Read the model definition and answer for the solid it produces. Units are mm, in the model's axes. A direction names the side the tool comes from. Give positions to 0.01 mm unless a question says otherwise; leave off trailing zeros. Write each loop counter-clockwise with the first axis right and the second up, starting at its lowest first coordinate (ties: lowest second). Pieces come first, ordered by that corner, then holes. Notation, with made-up numbers: M -23,-9 L 7,-9 A29 cw 7,22 Z; hole C 29.5,-27.5 d7. An arc over 180 degrees is marked long. Use a Markdown table: item, result. Add a question column.
Item 1: For faces 4 (the flat face through (-28, -25, 6.4)), 5 (the flat face through (0, 1, 0)), determine the directions among +Z, -Z, +X, -X, +Y, -Y from which every point of the face is accessible in a straight line to the end or side of a thin tool.
Item 2: A cutting plane is placed at B-B on y = -21. Determine the outline of the cut face in (x, z).
Item 3: A cutting plane is placed at D-D on y = -33. Determine the outline of the cut face in (x, z), then the cut area to 3 significant figures.
Item 4: A cutting plane is placed at C-C on z = 2.5. Count the separate pieces of the cut face and the enclosed holes in it, then the cut area to 3 significant figures.
Item 5: Consider probe 1 along Y at (x, z) = (28, 8.65); probe 2 along Y at (x, z) = (-28, 3); probe 3 along X at (y, z) = (19, 3.25). Determine where each line is inside the solid, lowest interval first. Write a range as [from, to].
Item 6: Given P1, Ø4.5, axis at x = 28, y = -33, coming from the -Z side; P2, Ø3.5, axis at x = -26, y = 22.5, coming from the -Z side; P3, Ø12, axis at x = 26, y = 19.5, coming from the -Z side, each flat-ended and moving along its own axis, determine where each tip first touches the part or whether it passes through.
Item 7: The mould has two halves that part along Y. Classify faces 1 (the flat face through (0, 1, 12)), 2 (the cylindrical face through (27.67, -30.52, 6.08)), 3 (the flat face through (0, -40, 6)): pulls with the +Y half, pulls with the -Y half, needs draft (parallel to the pull), parting line crosses it, or undercut.
Item 8: A cutting plane is placed at A-A on x = 28. Determine the outline of the cut face in (y, z), then the cut area to 3 significant figures.
from build123d import *

# Parameters (mm, degrees)
SKETCH_1_W                     = 70
SKETCH_1_H                     = 80
EXTRUDE_1_DEPTH                = 12
HOLE_WIZARD_M6_1_D             = 5
HOLE_WIZARD_M6_1_2_D           = 6.6
HOLE_WIZARD_M6_1_2_CBORE_D     = 11
HOLE_WIZARD_M6_1_2_CBORE_DEPTH = 6.4


with BuildPart() as part:
    # 草图1 → 凸台-拉伸1 (new body)
    with BuildSketch(Plane.XY):
        Rectangle(SKETCH_1_W, SKETCH_1_H)
    extrude(amount=EXTRUDE_1_DEPTH)

    # Hole Wizard M6 _1 (through all)
    with Locations(Plane(origin=(0, 0, 0), x_dir=(-1, 0, 0), z_dir=(0, 0, -1))):
        with Locations((28, 33), (28, -33), (-28, -33), (-28, 33)):
            Hole(HOLE_WIZARD_M6_1_D / 2)

    # Hole Wizard M6 _1 2 (through all)
    with Locations(Plane(origin=(0, 0, 0), x_dir=(-1, 0, 0), z_dir=(0, 0, -1))):
        with Locations((-28, -21), (-28, 21), (28, -21), (28, 21)):
            CounterBoreHole(HOLE_WIZARD_M6_1_2_D / 2, HOLE_WIZARD_M6_1_2_CBORE_D / 2, HOLE_WIZARD_M6_1_2_CBORE_DEPTH)


solid = part.part
Filled in:
| question | item | result |
|---|---|---|
| 1 | face 4 | -Z |
| 1 | face 5 | -Z, +X, -X, +Y, -Y |
| 2 | outline | M -35,0 L -33.5,0 L -33.5,6.4 L -31.3,6.4 L -31.3,12 L -35,12 Z; M -24.7,6.4 L -22.5,6.4 L -22.5,0 L 22.5,0 L 22.5,6.4 L 24.7,6.4 L 24.7,12 L -24.7,12 Z; M 31.3,6.4 L 33.5,6.4 L 33.5,0 L 35,0 L 35,12 L 31.3,12 Z |
| 3 | outline | M -35,0 L -30.5,0 L -30.5,12 L -35,12 Z; M -25.5,0 L 25.5,0 L 25.5,12 L -25.5,12 Z; M 30.5,0 L 35,0 L 35,12 L 30.5,12 Z |
| 3 | area | 720 mm² |
| 4 | separate pieces | 1 |
| 4 | enclosed holes | 8 |
| 4 | area | 5,140 mm² |
| 5 | probe 1 | [-40, -35.5], [-30.5, -24.3], [-17.7, 17.7], [24.3, 30.5], [35.5, 40] |
| 5 | probe 2 | [-40, -35.5], [-30.5, -26.5], [-15.5, 15.5], [26.5, 30.5], [35.5, 40] |
| 5 | probe 3 | [-35, -33.12], [-22.88, 22.88], [33.12, 35] |
| 6 | P1 | through |
| 6 | P2 | z = 6.4 |
| 6 | P3 | z = 0 |
| 7 | face 1 | needs draft |
| 7 | face 2 | undercut |
| 7 | face 3 | pulls with the -Y half |
| 8 | outline | M -40,0 L -35.5,0 L -35.5,12 L -40,12 Z; M -30.5,0 L -26.5,0 L -26.5,6.4 L -24.3,6.4 L -24.3,12 L -30.5,12 Z; M -17.7,6.4 L -15.5,6.4 L -15.5,0 L 15.5,0 L 15.5,6.4 L 17.7,6.4 L 17.7,12 L -17.7,12 Z; M 24.3,6.4 L 26.5,6.4 L 26.5,0 L 30.5,0 L 30.5,12 L 24.3,12 Z; M 35.5,0 L 40,0 L 40,12 L 35.5,12 Z |
| 8 | area | 625 mm² |
